Source: CAD feature listing. Evaluate the final solid. Frame: model axes, mm. A direction names the side the tool comes from. Give positions to 0.01 mm unless a question says otherwise; leave off trailing zeros. Loops run counter-clockwise (first coordinate to the right, second up) from the corner with the lowest first, then second, coordinate; pieces in that order, holes last. Notation, with made-up numbers: M 41,63.5 L 77,63.5 A20 cw 77,86.5 Z; hole C 39,69.25 d8. An arc over 180 degrees is marked long. Answer in a Markdown table with one row per item.
```python
from build123d import *

# Parameters (mm, degrees)
BOSS_EXTRUDE1_DEPTH = 1024


with BuildPart() as part:
    # Sketch1 → Boss-Extrude1 (new body)
    with BuildSketch(Plane.XY):
        with BuildLine():
            Line((0, 0), (30, 0))
            Line((30, 0), (30, 1))
            ThreePointArc((30, 1), (29.414213562, 2.414213562), (28, 3))
            Line((28, 3), (5, 3))
            ThreePointArc((5, 3), (3.585786438, 3.585786438), (3, 5))
            Line((3, 5), (3, 28))
            ThreePointArc((3, 28), (2.414213562, 29.414213562), (1, 30))
            Line((1, 30), (0, 30))
            Line((0, 30), (0, 0))
        make_face()
    extrude(amount=BOSS_EXTRUDE1_DEPTH)


solid = part.part
```
Q1. Ray query, probe 1 along Y at (x, z) = (16.75, 655); probe 2 along X at (y, z) = (4.25, 266). Return the intervals inside material, ascending. Write a range as from..to.
Values follow:
| item | result |
|---|---|
| probe 1 | 0..3 |
| probe 2 | 0..3.15 |
Q2. Reachability of faces 1 (the flat face through (0, 15, 505)), 2 (the flat face through (3, 16, 505)) from +Z, -Z, +X, -X, +Y, -Y: full face, straight path, thin tool, end or side. Return the list, or none.
Values follow:
| item | result |
|---|---|
| face 1 | +Z, -Z, -X, +Y, -Y |
| face 2 | +Z, -Z, +X, +Y |
Q3. Section query A-A (z = 859.5). Output: boundary loops of the cut face in (x, y), plus the area to 3 significant figures.
Values follow:
| item | result |
|---|---|
| outline | M 0,0 L 30,0 L 30,1 A2 ccw 28,3 L 5,3 A2 cw 3,5 L 3,28 A2 ccw 1,30 L 0,30 Z |
| area | 170 mm^2 |
Q4. Contact query for flat-ended pins moving along their axis: pin 1 Ø5 at (x, z) = (4.5, 729) entering from +Y; pin 2 Ø7 at (x, z) = (17.5, 383.5) entering from +Y; pin 3 Ø5 at (y, z) = (15, 791) entering from +X. Output: stop coordinate, or through.
Values follow:
| item | result |
|---|---|
| pin 1 | y = 29.73 |
| pin 2 | y = 3 |
| pin 3 | x = 3 |
Q5. Section query B-B (x = 11.75). Output: boundary loops of the cut face in (y, z), plus the area to 3 significant figures.
Values follow:
| item | result |
|---|---|
| outline | M 0,0 L 3,0 L 3,1024 L 0,1024 Z |
| area | 3,070 mm^2 |
